from build123d import *


with BuildPart() as part:
    # 草图2 → 旋转1 (revolve)
    with BuildSketch(Plane(origin=(0, 0, 0), x_dir=(0, 0, -1), z_dir=(1, 0, 0))):
        with BuildLine():
            Line((-22.9, 9), (-18.138357147, 9))
            ThreePointArc((-18.138357147, 9), (-20.248456731, 0), (-18.138357147, -9))
            Line((-18.138357147, -9), (-22.9, -9))
            ThreePointArc((-22.9, -9), (-23.324264069, -8.824264069), (-23.5, -8.4))
            Line((-23.5, -8.4), (-23.5, 8.4))
            ThreePointArc((-23.5, 8.4), (-23.324264069, 8.824264069), (-22.9, 9))
        make_face()
    revolve(axis=Axis((0, 11, 0), (0, -1, 0)))

    # 草图3 → 旋转2 (revolve)
    with BuildSketch(Plane(origin=(0, 0, 0), x_dir=(0, 0, -1), z_dir=(1, 0, 0))):
        with BuildLine():
            Line((-16.670388475, 11), (-15, 11))
            Line((-15, 11), (-15, -11))
            Line((-15, -11), (-16.670388475, -11))
            ThreePointArc((-16.670388475, -11), (-16.961464654, -10.924666235), (-17.179447951, -10.717582194))
            ThreePointArc((-17.179447951, -10.717582194), (-20.248456731, 0), (-17.179447951, 10.717582194))
            ThreePointArc((-17.179447951, 10.717582194), (-16.961464654, 10.924666235), (-16.670388475, 11))
        make_face()
    revolve(axis=Axis((0, 11, 0), (0, -1, 0)))


solid = part.part
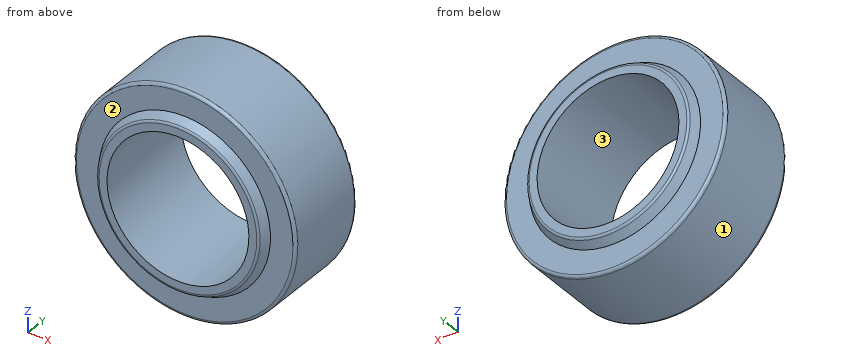
The model under review builds one solid part; all positions refer to its coordinate system, in mm. Face numbers are marked on the shaded views. Give positions to 0.01 mm unless a question says otherwise; leave off trailing zeros. Order: outer loops, then holes, each group sorted by start corner. A loop starts at its lowest first (then second) coordinate and runs counter-clockwise, first axis right, second up. Notation, with made-up numbers: (32, -34.75) -> (87, -34.75) arc R32 ccw to (87, 0.25) -> close; hole circle Ø10 at (69.25, -33). An arc over 180 degrees is marked (long way). Write item = value, one per line. Start each with the question number.
(1) Draft analysis for pull direction X (two halves, no side actions). For the marked faces 1, 2 and 3, state which applies: +X half, -X half, draft (parallel to the pull), parting line (faces both ways), or undercut.
(2) Take a section at A-A (z = 0). Write out the cut boundary in (x, y).
(3) For pin 1 Ø2 at (y, z) = (4, -3) entering from +X; pin 2 Ø2 at (x, z) = (14, -1) entering from +Y; pin 3 Ø3 at (x, z) = (-0.5, -13) entering from -Y; pin 4 Ø10 at (x, y) = (16, -2.5) entering from +Z, all flat-tipped, find the tip position at first contact; note any pin that passes through.
(4) Take a section at B-B (x = 0). Write out the cut boundary in (y, z), plus the area to 3 significant figures.
(5) For L1, parallel to Z at x = 0, y = -3.25; L2, parallel to X at y = -7.25, z = 11, list the stretches that pass through material, from the lowest coordinate up. Write a range as from..to.
(6) Take a section at C-C (y = 7). Write out the cut boundary in (x, z).
Returned:
q1.face_1 = parting line
q1.face_2 = draft
q1.face_3 = undercut
q2.outline = (-23.5, -8.4) arc R0.6 ccw to (-22.9, -9) -> (-18.14, -9) arc R20.25 ccw to (-17.18, -10.72) arc R0.6 ccw to (-16.67, -11) -> (-15, -11) -> (-15, 11) -> (-16.67, 11) arc R0.6 ccw to (-17.18, 10.72) arc R20.25 ccw to (-18.14, 9) -> (-22.9, 9) arc R0.6 ccw to (-23.5, 8.4) -> close; (15, -11) -> (16.67, -11) arc R0.6 ccw to (17.18, -10.72) arc R20.25 ccw to (18.14, -9) -> (22.9, -9) arc R0.6 ccw to (23.5, -8.4) -> (23.5, 8.4) arc R0.6 ccw to (22.9, 9) -> (18.14, 9) arc R20.25 ccw to (17.18, 10.72) arc R0.6 ccw to (16.67, 11) -> (15, 11) -> close
q3.pin_1 = 23.41
q3.pin_2 = 11
q3.pin_3 = through
q3.pin_4 = 20.77
q4.outline = (-11, -16.67) arc R0.6 ccw to (-10.72, -17.18) arc R20.25 ccw to (-9, -18.14) -> (-9, -22.9) arc R0.6 ccw to (-8.4, -23.5) -> (8.4, -23.5) arc R0.6 ccw to (9, -22.9) -> (9, -18.14) arc R20.25 ccw to (10.72, -17.18) arc R0.6 ccw to (11, -16.67) -> (11, -15) -> (-11, -15) -> close; (-11, 15) -> (11, 15) -> (11, 16.67) arc R0.6 ccw to (10.72, 17.18) arc R20.25 ccw to (9, 18.14) -> (9, 22.9) arc R0.6 ccw to (8.4, 23.5) -> (-8.4, 23.5) arc R0.6 ccw to (-9, 22.9) -> (-9, 18.14) arc R20.25 ccw to (-10.72, 17.18) arc R0.6 ccw to (-11, 16.67) -> close
q4.area = 326 mm²
q5.L1 = -23.5..-15, 15..23.5
q5.L2 = -20.77..-10.2, 10.2..20.77
q6.outline = circle Ø47 at (0, 0); hole circle Ø30 at (0, 0)
